from build123d import *

# Parameters (mm, degrees)
SKETCH_1_W                = 55
SKETCH_1_H                = 148
EXTRUDE_1_DEPTH           = 6
CHAMFER_1_SIZE            = 3
HOLE_WIZARD_1_D           = 4.5
HOLE_WIZARD_1_CBORE_D     = 8
HOLE_WIZARD_1_CBORE_DEPTH = 4.6
HOLE_WIZARD_M6_1_D        = 5
HOLE_WIZARD_M6_1_DEPTH    = 15
HOLE_WIZARD_M6_1_TIP      = 1.502151548
HOLE_WIZARD_2_D           = 5.5
HOLE_WIZARD_2_CBORE_D     = 10
HOLE_WIZARD_2_CBORE_DEPTH = 5.7


with BuildPart() as part:
    # 草图1 → 凸台-拉伸1 (new, symmetric)
    with BuildSketch(Plane(origin=(0, 0, 0), x_dir=(1, 0, 0), z_dir=(0, 1, 0))):
        Rectangle(SKETCH_1_W, SKETCH_1_H)
    extrude(amount=EXTRUDE_1_DEPTH, both=True)

    # 倒角1
    chamfer_1_edges = [part.edges().sort_by_distance(p)[0] for p in [
        (-27.5, 0, -74),
        (27.5, 0, -74),
    ]]
    chamfer(chamfer_1_edges, length=CHAMFER_1_SIZE)

    # 打孔尺寸(%根据)内六角圆柱头螺钉的类型1 (through all)
    with Locations(Plane(origin=(0, 6, 0), x_dir=(1, 0, 0), z_dir=(0, 1, 0))):
        with Locations((13, 41.5), (13, 67.5), (-13, 67.5), (-13, 41.5)):
            CounterBoreHole(HOLE_WIZARD_1_D / 2, HOLE_WIZARD_1_CBORE_D / 2, HOLE_WIZARD_1_CBORE_DEPTH)

    # M6 螺纹孔1
    with Locations(Plane.XY.offset(74)):
        with Locations((20, 0), (-20, 0)):
            Hole(HOLE_WIZARD_M6_1_D / 2, depth=HOLE_WIZARD_M6_1_DEPTH)
            with Locations((0, 0, -(HOLE_WIZARD_M6_1_DEPTH + HOLE_WIZARD_M6_1_TIP / 2))):  # 118° drill point
                Cone(0, HOLE_WIZARD_M6_1_D / 2, HOLE_WIZARD_M6_1_TIP, mode=Mode.SUBTRACT)

    # 打孔尺寸(%根据)内六角圆柱头螺钉的类型2 (through all)
    with Locations(Plane.XZ.offset(6)):
        with Locations((0, 59), (0, -21)):
            CounterBoreHole(HOLE_WIZARD_2_D / 2, HOLE_WIZARD_2_CBORE_D / 2, HOLE_WIZARD_2_CBORE_DEPTH)


solid = part.part
Work out the finished part from the listing and answer in its coordinate system (mm). A direction names the side the tool comes from. Give positions to 0.01 mm unless a question says otherwise; leave off trailing zeros. Write each loop counter-clockwise with the first axis right and the second up, starting at its lowest first coordinate (ties: lowest second). Pieces come first, ordered by that corner, then holes.
Q1. The part is cut by section C-C on y = 4.5. Give the vertices of the cut face in (x, z).
Answer:
outline: (-27.5, -71) - (-24.5, -74) - (24.5, -74) - (27.5, -71) - (27.5, 74) - (-27.5, 74) - close; hole circle Ø8 at (-13, -67.5); hole circle Ø8 at (-13, -41.5); hole circle Ø5.5 at (0, -21); hole circle Ø5.5 at (0, 59); hole circle Ø8 at (13, -67.5); hole circle Ø8 at (13, -41.5)
Q2. The part is cut by section B-B on x = -13. Give the vertices of the cut face in (y, z), and give its area (3 significant figures).
Answer:
outline: (-6, -74) - (6, -74) - (6, -71.5) - (1.4, -71.5) - (1.4, -69.75) - (-6, -69.75) - close; (-6, -65.25) - (1.4, -65.25) - (1.4, -63.5) - (6, -63.5) - (6, -45.5) - (1.4, -45.5) - (1.4, -43.75) - (-6, -43.75) - close; (-6, -39.25) - (1.4, -39.25) - (1.4, -37.5) - (6, -37.5) - (6, 74) - (-6, 74) - close
area: 1,640 mm2
Q3. The part is cut by section D-D on y = -4.5. Give the vertices of the cut face in (x, z).
Answer:
outline: (-27.5, -71) - (-24.5, -74) - (24.5, -74) - (27.5, -71) - (27.5, 74) - (-27.5, 74) - close; hole circle Ø4.5 at (-13, -67.5); hole circle Ø4.5 at (-13, -41.5); hole circle Ø10 at (0, -21); hole circle Ø10 at (0, 59); hole circle Ø4.5 at (13, -67.5); hole circle Ø4.5 at (13, -41.5)
Q4. The part is cut by section A-A on z = -41.5. Give the vertices of the cut face in (x, y).
Answer:
outline: (-27.5, -6) - (-15.25, -6) - (-15.25, 1.4) - (-17, 1.4) - (-17, 6) - (-27.5, 6) - close; (-10.75, -6) - (10.75, -6) - (10.75, 1.4) - (9, 1.4) - (9, 6) - (-9, 6) - (-9, 1.4) - (-10.75, 1.4) - close; (15.25, -6) - (27.5, -6) - (27.5, 6) - (17, 6) - (17, 1.4) - (15.25, 1.4) - close
Q5. Given pin 1 (6.5 mm diameter, centred on x = -13, z = -41.5, fed in from +Y); pin 2 (3 mm diameter, centred on x = -1, z = -20, fed in from -Y); pin 3 (3.5 mm diameter, centred on x = -13, z = -67.5, fed in from +Y), each flat-ended and moving along its own axis, determine where each tip first touches the part or whether it passes through.
Answer:
pin 1: stops at y = 1.4
pin 2: stops at y = -0.3
pin 3: passes through
Q6. Straight lines are drawn through the part: L1, parallel to Z at x = 0, y = 1.5; L2, parallel to Z at x = 13, y = -4; L3, parallel to X at y = -2.75, z = -67.5. For each, find the intervals that lie inside material, in ascending order.
Answer:
L1: z = -74 to -23.75, -18.25 to 56.25, 61.75 to 74
L2: z = -74 to -69.75, -65.25 to -43.75, -39.25 to 74
L3: x = -27.5 to -15.25, -10.75 to 10.75, 15.25 to 27.5
Q7. For a pull along X with two mould halves and no side action, classify faces 4 (the face through (-13.867, 3.732, -63.595)), 5 (the face through (0, 0, -74)), 6 (the face through (-27.5, 0, 3)) as released by +X, released by -X, zero draft, split by the parting line, or undercut.
Answer:
face 4: undercut
face 5: zero draft
face 6: released by -X
Q8. A tool of negligible diameter and unlimited length cuts with its end or side. For faces 1 (the face through (15, 1.4, -66)), 2 (the face through (-26, 0.1, -72.5)), 3 (the face through (-0.651, -3.19, 63.957)), from which of +Z, -Z, +X, -X, +Y, -Y can it reach the whole face along a straight path? Write none if from no direction.
Answer:
face 1: +Y
face 2: -Z, -X, +Y, -Y
face 3: -Y
